from build123d import *

# Parameters (mm, degrees)
EXTRUDE_1_DEPTH     = 25
CUT_EXTRUDE_1_DEPTH = 10
CUT_EXTRUDE_2_DEPTH = 10
FILLET_1_R          = 3
FILLET_2_R          = 1
FILLET_3_R          = 3


with BuildPart() as part:
    # 草图9 → 拉伸-薄壁1 (new, symmetric)
    with BuildSketch(Plane.XY):
        Polygon((17, 0), (0, 0), (0, 15), (-2, 15), (-2, -2), (17, -2), align=None)
    extrude(amount=EXTRUDE_1_DEPTH, both=True)

    # 草图10 → 切除-拉伸1 (cut)
    with BuildSketch(Plane(origin=(0, 0, 0), x_dir=(1, 0, 0), z_dir=(0, 1, 0))):
        with BuildLine():
            Line((9, 21.75), (13, 21.75))
            ThreePointArc((13, 21.75), (14.75, 20), (13, 18.25))
            Line((13, 18.25), (9, 18.25))
            ThreePointArc((9, 18.25), (7.25, 20), (9, 21.75))
        make_face()
        with BuildLine():
            Line((9, -21.75), (13, -21.75))
            ThreePointArc((13, -21.75), (14.75, -20), (13, -18.25))
            Line((13, -18.25), (9, -18.25))
            ThreePointArc((9, -18.25), (7.25, -20), (9, -21.75))
        make_face()
        with BuildLine():
            Line((9, 1.75), (13, 1.75))
            ThreePointArc((13, 1.75), (14.75, 0), (13, -1.75))
            Line((13, -1.75), (9, -1.75))
            ThreePointArc((9, -1.75), (7.25, 0), (9, 1.75))
        make_face()
    extrude(amount=-CUT_EXTRUDE_1_DEPTH, mode=Mode.SUBTRACT)

    # 草图11 → 切除-拉伸2 (cut)
    with BuildSketch(Plane(origin=(0, 0, 0), x_dir=(0, 0, -1), z_dir=(1, 0, 0))):
        with BuildLine():
            Line((-10.75, 10.5), (-10.75, 6.5))
            ThreePointArc((-10.75, 6.5), (-12.5, 4.75), (-14.25, 6.5))
            Line((-14.25, 6.5), (-14.25, 10.5))
            ThreePointArc((-14.25, 10.5), (-12.5, 12.25), (-10.75, 10.5))
        make_face()
        with BuildLine():
            Line((10.75, 10.5), (10.75, 6.5))
            ThreePointArc((10.75, 6.5), (12.5, 4.75), (14.25, 6.5))
            Line((14.25, 6.5), (14.25, 10.5))
            ThreePointArc((14.25, 10.5), (12.5, 12.25), (10.75, 10.5))
        make_face()
    extrude(amount=-CUT_EXTRUDE_2_DEPTH, mode=Mode.SUBTRACT)

    # 圆角1
    fillet_1_edges = [part.edges().sort_by_distance(p)[0] for p in [
        (-1, 15, 25),
        (-1, 15, -25),
        (17, -1, -25),
        (17, -1, 25),
    ]]
    fillet(fillet_1_edges, radius=FILLET_1_R)

    # 圆角2
    fillet_2_edges = [part.edges().sort_by_distance(p)[0] for p in [
        (0, 0, 0),
    ]]
    fillet(fillet_2_edges, radius=FILLET_2_R)

    # 圆角3
    fillet_3_edges = [part.edges().sort_by_distance(p)[0] for p in [
        (-2, -2, 0),
    ]]
    fillet(fillet_3_edges, radius=FILLET_3_R)


solid = part.part
Design review of the part built by this model. Coordinates are the model's own, in mm. A direction names the side the tool comes from. Round coordinates to 2 decimals unless told otherwise and drop trailing zeros. Write each loop counter-clockwise with the first axis right and the second up, starting at its lowest first coordinate (ties: lowest second). Pieces come first, ordered by that corner, then holes. Notation, with made-up numbers: (-21.5, 49.25) - (18.5, 49.25) arc R28 cw to (18.5, 77.25) - close; hole circle Ø8 at (-13.75, 40.25). An arc over 180 degrees is marked (long way). Return JSON: item names as keys, results as strings. Group by question number.
Item 1: Machinability: for faces 1 (the face through (16.1, -0.99, -24.14)), 2 (the face through (0, 8, 0)), 3 (the face through (14.75, -0.99, -0.04)), 4 (the face through (-0.99, 12.25, -12.54)), which of the approach directions +Z, -Z, +X, -X, +Y, -Y give a long, thin tool a straight path to every point of the face, cutting with its end or side? Answer none if there is none.
Item 2: For probe 1 along Y at (x, z) = (13.5, 5); probe 2 along X at (y, z) = (-0.5, 15), list the stretches that pass through material, from the lowest coordinate up. Write a range as [from, to].
Item 3: Insertion check: P1, Ø5, axis at x = 10, z = 5.5, coming from the +Y side; P2, Ø6, axis at y = 13, z = -18, coming from the +X side; P3, Ø6, axis at x = 3.5, y = 13, coming from the -Z side; P4, Ø8, axis at x = 10, y = 3.5, coming from the -Z side. Each pin has a flat end and moves straight along its axis. Give the tip position at first contact, or say it passes through.
Item 4: The part is to be moulded in two halves that separate along X. For faces 5 (the face through (-0.99, 4.75, 12.46)), 6 (the face through (-1.1, -1.14, -0.35)), 7 (the face through (11, -1, -18.25)), say which applies: pulls with the +X half, pulls with the -X half, needs draft (parallel to the pull), parting line crosses it, or undercut.
Item 5: We need section C-C on z = -12.5. Write out the cut boundary in (x, y).
Item 6: We need section B-B on x = 11. Write out the cut boundary in (y, z), and give its area (3 significant figures).
Item 7: We need section D-D on x = -1. Write out the cut boundary in (y, z).
Item 8: We need section A-A on y = 9.75. Write out the cut boundary in (x, z).
Model answer:
{
 "1": {"face 1": "-Z, +X, +Y, -Y", "face 2": "+Z, -Z, +X, +Y", "face 3": "+Y, -Y", "face 4": "+X, -X"},
 "2": {"probe 1": "y = [-2, 0]", "probe 2": "x = [-1.6, 17]"},
 "3": {"P1": "stops at y = 0", "P2": "stops at x = 0", "P3": "passes through", "P4": "stops at z = -25"},
 "4": {"face 5": "needs draft", "face 6": "pulls with the -X half", "face 7": "undercut"},
 "5": {"outline": "(-2, 1) arc R3 ccw to (1, -2) - (17, -2) - (17, 0) - (1, 0) arc R1 cw to (0, 1) - (0, 4.75) - (-2, 4.75) - close; (-2, 12.25) - (0, 12.25) - (0, 15) - (-2, 15) - close"},
 "6": {"outline": "(-2, -25) - (0, -25) - (0, -21.75) - (-2, -21.75) - close; (-2, -18.25) - (0, -18.25) - (0, -1.75) - (-2, -1.75) - close; (-2, 1.75) - (0, 1.75) - (0, 18.25) - (-2, 18.25) - close; (-2, 21.75) - (0, 21.75) - (0, 25) - (-2, 25) - close", "area": "79.0 mm²"},
 "7": {"outline": "(-1.24, -25) - (12, -25) arc R3 ccw to (15, -22) - (15, 22) arc R3 ccw to (12, 25) - (-1.24, 25) - close; hole (6.5, -14.25) - (10.5, -14.25) arc R1.75 ccw to (10.5, -10.75) - (6.5, -10.75) arc R1.75 ccw to start; hole (6.5, 10.75) - (10.5, 10.75) arc R1.75 ccw to (10.5, 14.25) - (6.5, 14.25) arc R1.75 ccw to start"},
 "8": {"outline": "(-2, -25) - (0, -25) - (0, -14.25) - (-2, -14.25) - close; (-2, -10.75) - (0, -10.75) - (0, 10.75) - (-2, 10.75) - close; (-2, 14.25) - (0, 14.25) - (0, 25) - (-2, 25) - close"}
}
